from build123d import *

# Parameters (mm, degrees)
SKETCH1_R           = 6.25
BOSS_EXTRUDE1_DEPTH = 4.5


with BuildPart() as part:
    # Sketch1 → Boss-Extrude1 (new body)
    with BuildSketch(Plane.XY):
        with BuildLine():
            Line((25, 85), (5, 85))
            ThreePointArc((5, 85), (1.464466094, 83.535533906), (0, 80))
            Line((0, 80), (0, 20))
            ThreePointArc((0, 20), (5.857864376, 5.857864376), (20, 0))
            Line((20, 0), (55, 0))
            ThreePointArc((55, 0), (58.535533906, 1.464466094), (60, 5))
            Line((60, 5), (60, 30))
            ThreePointArc((60, 30), (58.535533906, 33.535533906), (55, 35))
            Line((55, 35), (50, 35))
            ThreePointArc((50, 35), (35.857864376, 40.857864376), (30, 55))
            Line((30, 55), (30, 80))
            ThreePointArc((30, 80), (28.535533906, 83.535533906), (25, 85))
        make_face()
        with Locations((15, 40)):
            Circle(SKETCH1_R, mode=Mode.SUBTRACT)
        with Locations((15, 70)):
            Circle(SKETCH1_R, mode=Mode.SUBTRACT)
    extrude(amount=BOSS_EXTRUDE1_DEPTH)


solid = part.part
Here's how the part is built. I have some questions about the finished solid (model axes, mm). A direction names the side the tool comes from. Coordinates: 2 decimals unless noted, no trailing zeros. Order: outer loops, then holes, each group sorted by start corner. A loop starts at its lowest first (then second) coordinate and runs counter-clockwise, first axis right, second up. Notation, with made-up numbers: (49.25, 51.5) -> (93.25, 51.5) arc R19 ccw to (93.25, 59.5) -> close; hole circle Ø2 at (79.25, -1). An arc over 180 degrees is marked (long way). Answer in a Markdown table with one row per item.
(1) Thinking about a two-plate mould opening in Y: for faces 1 (the face through (14.2, 76.2, 2.2)), 2 (the face through (23, 34, 4.5)), 3 (the face through (15, 85, 2)), which applies, +Y half, -Y half, draft (parallel to the pull), parting line (faces both ways), or undercut?
Answer key:
| item | result |
|---|---|
| face 1 | undercut |
| face 2 | draft |
| face 3 | +Y half |
(2) On a 3-axis mill with a long thin cutter (end or side, diameter ignored), from which of +Z, -Z, +X, -X, +Y, -Y can I reach the whole of each face in a straight line? I mean faces 4 (the face through (0, 50, 2)), 5 (the face through (30, 67, 2)). Say none if no direction works.
Answer key:
| item | result |
|---|---|
| face 4 | +Z, -Z, -X, +Y, -Y |
| face 5 | +Z, -Z, +X, +Y |
(3) Please list where these lines run through material, in increasing order: probe 1 along Y at (x, z) = (11, 0.8); probe 2 along X at (y, z) = (59, 3); probe 3 along Y at (x, z) = (15, 1.2).
Answer key:
| item | result |
|---|---|
| probe 1 | 2.14 to 35.2, 44.8 to 65.2, 74.8 to 85 |
| probe 2 | 0 to 30 |
| probe 3 | 0.64 to 33.75, 46.25 to 63.75, 76.25 to 85 |
(4) I want a section at B-B on x = 15. List the corners of the cut face in (y, z) for me, then the cut area to 3 significant figures.
Answer key:
| item | result |
|---|---|
| outline | (0.64, 0) -> (33.75, 0) -> (33.75, 4.5) -> (0.64, 4.5) -> close; (46.25, 0) -> (63.75, 0) -> (63.75, 4.5) -> (46.25, 4.5) -> close; (76.25, 0) -> (85, 0) -> (85, 4.5) -> (76.25, 4.5) -> close |
| area | 267 mm^2 |
(5) Will these pins go through, and if not, where does the flat tip stop? pin 1 Ø7.5 at (x, y) = (15, 40) entering from -Z; pin 2 Ø1.5 at (y, z) = (72, 4) entering from +X; pin 3 Ø2 at (x, z) = (52.5, 1.5) entering from +Y; pin 4 Ø4 at (x, y) = (7, 13.5) entering from -Z.
Answer key:
| item | result |
|---|---|
| pin 1 | through |
| pin 2 | x = 30 |
| pin 3 | y = 35 |
| pin 4 | z = 0 |
(6) I want a section at A-A on y = 70. List the corners of the cut face in (x, z) for me.
Answer key:
| item | result |
|---|---|
| outline | (0, 0) -> (8.75, 0) -> (8.75, 4.5) -> (0, 4.5) -> close; (21.25, 0) -> (30, 0) -> (30, 4.5) -> (21.25, 4.5) -> close |
(7) I want a section at D-D on x = 52.5. List the corners of the cut face in (y, z) for me.
Answer key:
| item | result |
|---|---|
| outline | (0, 0) -> (35, 0) -> (35, 4.5) -> (0, 4.5) -> close |
(8) I want a section at C-C on z = 1.9. List the corners of the cut face in (x, y) for me.
Answer key:
| item | result |
|---|---|
| outline | (0, 20) arc R20 ccw to (20, 0) -> (55, 0) arc R5 ccw to (60, 5) -> (60, 30) arc R5 ccw to (55, 35) -> (50, 35) arc R20 cw to (30, 55) -> (30, 80) arc R5 ccw to (25, 85) -> (5, 85) arc R5 ccw to (0, 80) -> close; hole circle Ø12.5 at (15, 40); hole circle Ø12.5 at (15, 70) |
